The drawing under review shows one solid part. Ordinate dimensions are in mm from its lowest x, y, z. Give positions to 0.01 mm unless a question says otherwise; leave off trailing zeros. Write each loop counter-clockwise with the first axis right and the second up, starting at its lowest first coordinate (ties: lowest second). Pieces come first, ordered by that corner, then holes. Notation, with made-up numbers: M 57,15.25 L 113,15.25 A23 cw 113,33.25 Z; hole C 11.5,-19 d4. An arc over 180 degrees is marked long. Write item = value, one per line. Start each with the question number.
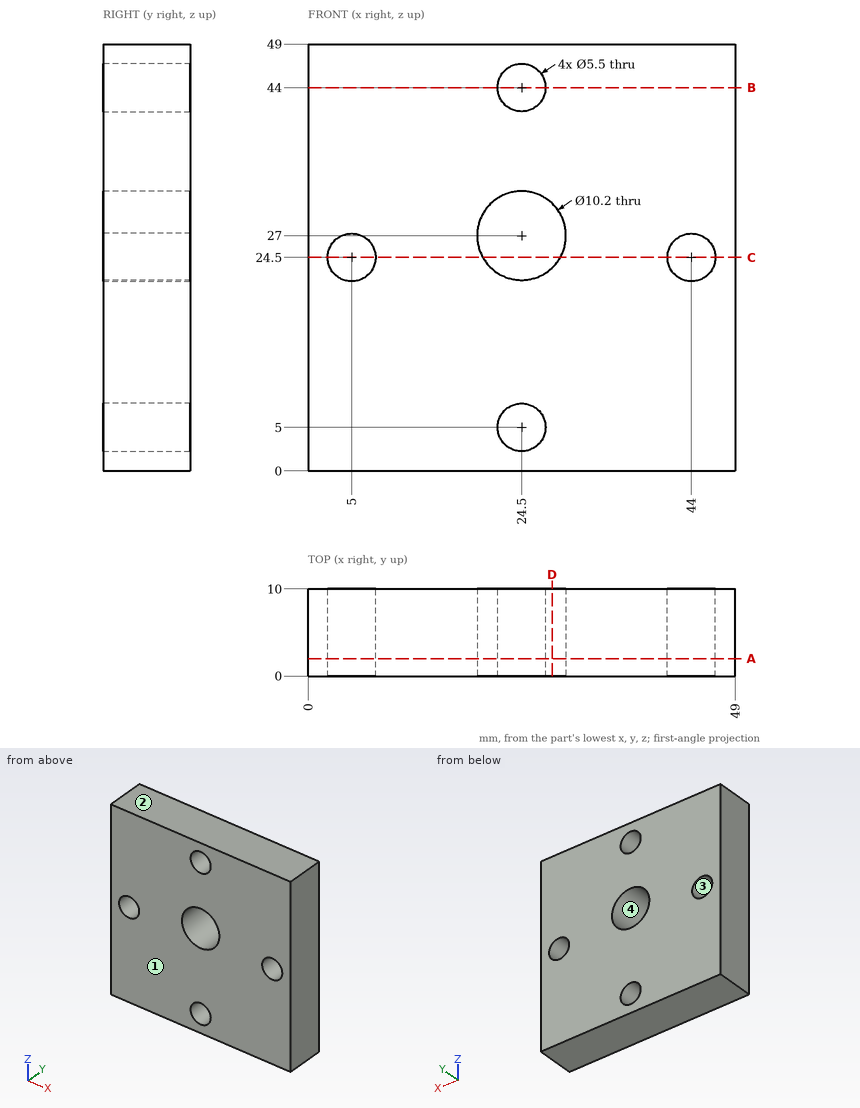
Item 1: Clearance check with a flat-ended pin moving along its axis: P1, Ø9, axis at x = 24.5, z = 44, coming from the +Y side. State where the tip first meets the part, or that it passes through.
Item 2: We need section B-B, the plane z = 44. Write out the cut boundary in (x, y), and give its area (3 significant figures).
Item 3: To check wall thickness, follow probe 1 along X at (y, z) = (6, 27); probe 2 along X at (y, z) = (4, 26); probe 3 along X at (y, z) = (3, 5). State the ranges of each line that lie inside material, in increasing order. Write a range as [from, to].
Item 4: We need section A-A, the plane y = 2. Write out the cut boundary in (x, z), and give its area (3 significant figures).
Item 5: We need section C-C, the plane z = 24.5. Write out the cut boundary in (x, y).
Item 6: The part is to be moulded in two halves that separate along Z. For the marked faces 1, 2, 3 and 4, say which applies: released by +Z, released by -Z, zero draft, split by the parting line, or undercut.
Item 7: We need section D-D, the plane x = 28. Write out the cut boundary in (y, z).
Worked out:
q1.P1 = 10
q2.outline = M 0,0 L 21.75,0 L 21.75,10 L 0,10 Z; M 27.25,0 L 49,0 L 49,10 L 27.25,10 Z
q2.area = 435 mm²
q3.probe_1 = [0, 3.85], [6.15, 19.4], [29.6, 42.85], [45.15, 49]
q3.probe_2 = [0, 2.7], [7.3, 19.5], [29.5, 41.7], [46.3, 49]
q3.probe_3 = [0, 21.75], [27.25, 49]
q4.outline = M 0,0 L 49,0 L 49,49 L 0,49 Z; hole C 5,24.5 d5.5; hole C 24.5,27 d10.2; hole C 24.5,5 d5.5; hole C 24.5,44 d5.5; hole C 44,24.5 d5.5
q4.area = 2,220 mm²
q5.outline = M 0,0 L 2.25,0 L 2.25,10 L 0,10 Z; M 7.75,0 L 20.05,0 L 20.05,10 L 7.75,10 Z; M 28.95,0 L 41.25,0 L 41.25,10 L 28.95,10 Z; M 46.75,0 L 49,0 L 49,10 L 46.75,10 Z
q6.face_1 = zero draft
q6.face_2 = released by +Z
q6.face_3 = undercut
q6.face_4 = undercut
q7.outline = M 0,0 L 10,0 L 10,23.29 L 0,23.29 Z; M 0,30.71 L 10,30.71 L 10,49 L 0,49 Z
